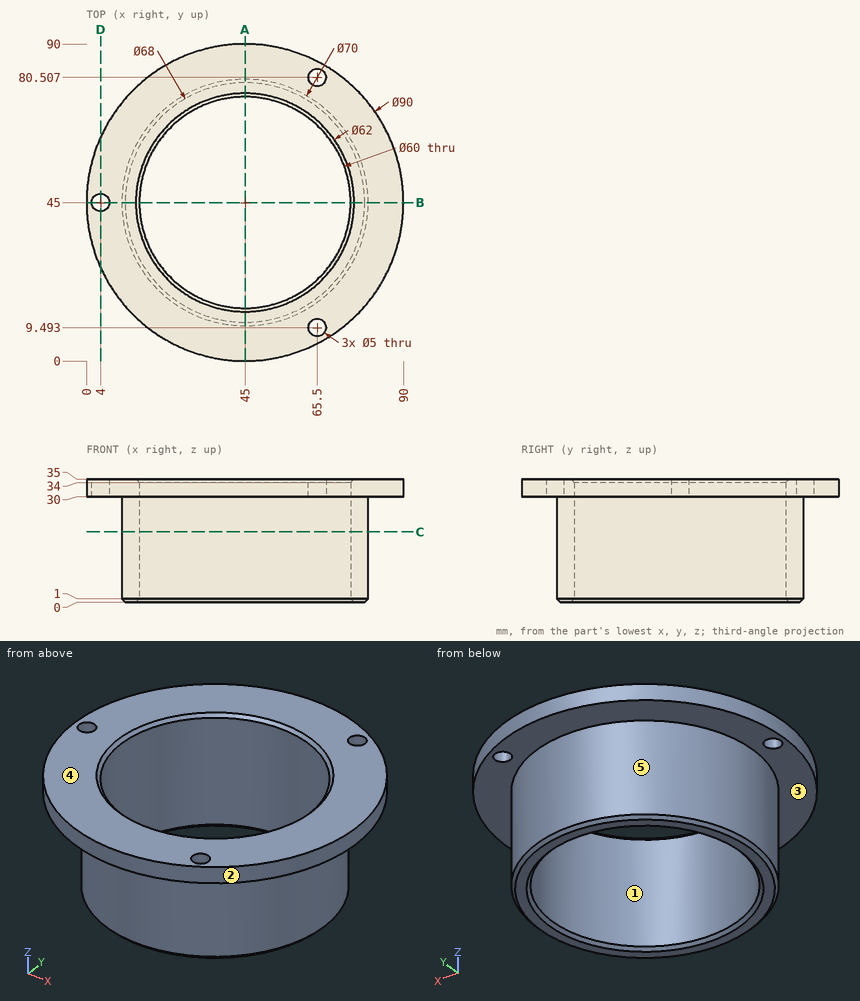
Verification items for this drawing (mm, ordinates from the low corner). A direction names the side the tool comes from. Coordinates: 2 decimals unless noted, no trailing zeros. Order: outer loops, then holes, each group sorted by start corner. A loop starts at its lowest first (then second) coordinate and runs counter-clockwise, first axis right, second up.
Q1. Depth check by flat-ended pin: pin 1 Ø10 at (x, z) = (62.5, 10) entering from -Y; pin 2 Ø1.5 at (y, z) = (50, 20.5) entering from -X; pin 3 Ø4 at (x, z) = (63.5, 10) entering from +Y; pin 4 Ø3 at (x, y) = (4, 45) entering from -Z. Enter the tip coordinate at first touch or a pass-through.
Reply:
pin 1: stops at y = 12.31
pin 2: stops at x = 10.26
pin 3: stops at y = 75.87
pin 4: passes through
Q2. Thickness scan on probe 1 along X at (y, z) = (45.5, 22); probe 2 along Z at (x, y) = (74, 16.5); probe 3 along Y at (x, z) = (65.5, 31.15). Record the ranges inside material, lowest first.
Reply:
probe 1: x = 10 to 15, 75 to 80
probe 2: z = 30 to 35
probe 3: y = 4.94 to 6.99, 11.99 to 23.1, 66.9 to 78.01, 83.01 to 85.06
Q3. Sectioned sample at A-A on x = 45. Record the cut outline in (y, z), and give its area (3 significant figures).
Reply:
outline: (0, 30) - (10, 30) - (10, 1) - (11, 0) - (14, 0) - (15, 1) - (15, 34) - (14, 35) - (0, 35) - close; (75, 1) - (76, 0) - (79, 0) - (80, 1) - (80, 30) - (90, 30) - (90, 35) - (76, 35) - (75, 34) - close
area: 447 mm2
Q4. Draft check along Y on the marked faces 1, 2 and 3. Enter one of: released by +Y, released by -Y, zero draft, split by the parting line, or undercut.
Reply:
face 1: undercut
face 2: split by the parting line
face 3: zero draft
Q5. Sectioned sample at B-B on y = 45. Record the cut outline in (x, z), and give its area (3 significant figures).
Reply:
outline: (0, 30) - (1.5, 30) - (1.5, 35) - (0, 35) - close; (6.5, 30) - (10, 30) - (10, 1) - (11, 0) - (14, 0) - (15, 1) - (15, 34) - (14, 35) - (6.5, 35) - close; (75, 1) - (76, 0) - (79, 0) - (80, 1) - (80, 30) - (90, 30) - (90, 35) - (76, 35) - (75, 34) - close
area: 422 mm2
Q6. Sectioned sample at C-C on z = 20. Record the cut outline in (x, y).
Reply:
outline: circle Ø70 at (45, 45); hole circle Ø60 at (45, 45)
Q7. Sectioned sample at D-D on x = 4. Record the cut outline in (y, z).
Reply:
outline: (26.45, 30) - (42.5, 30) - (42.5, 35) - (26.45, 35) - close; (47.5, 30) - (63.55, 30) - (63.55, 35) - (47.5, 35) - close
Q8. Tool access check on the marked faces 4 and 5. Record the directions out of +Z, -Z, +X, -X, +Y, -Y that give a thin tool (end or side, any length) a straight path to the whole face; none if there is none.
Reply:
face 4: +Z, +X, -X, +Y, -Y
face 5: -Z
